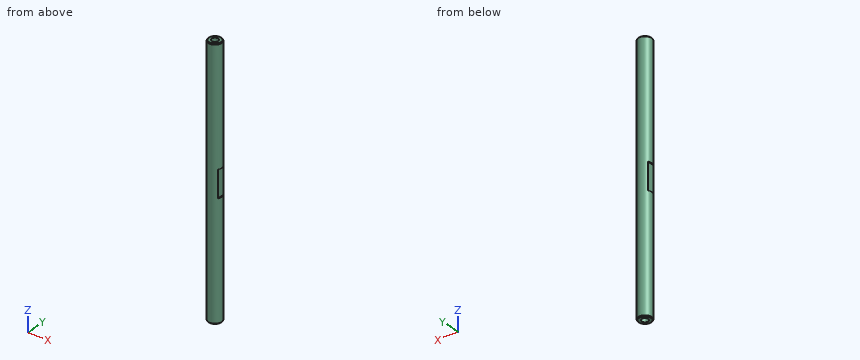
```python
from build123d import *

# Parameters (mm, degrees)
SKETCH_1_R             = 5
EXTRUDE_1_DEPTH        = 97
CUT_EXTRUDE_1_DEPTH    = 10
HOLE_WIZARD_M6_1_D     = 5
HOLE_WIZARD_M6_1_DEPTH = 15
HOLE_WIZARD_M6_1_TIP   = 1.502151548
HOLE_WIZARD_M6_2_D     = 5
HOLE_WIZARD_M6_2_DEPTH = 15
HOLE_WIZARD_M6_2_TIP   = 1.502151548
CHAMFER_1_SIZE         = 0.5


with BuildPart() as part:
    # 草图1 → 凸台-拉伸1 (new, symmetric)
    with BuildSketch(Plane.XY):
        with Locations(Location((0, 0, 0), (0, 0, 180))):
            Circle(SKETCH_1_R)
    extrude(amount=EXTRUDE_1_DEPTH, both=True)

    # 草图2 → 切除-拉伸1 (cut, symmetric)
    with BuildSketch(Plane.XY):
        with BuildLine():
            Line((-4.25, 2.633913438), (-4.25, -2.633913438))
            ThreePointArc((-4.25, -2.633913438), (-5, 0), (-4.25, 2.633913438))
        make_face()
        with BuildLine():
            Line((4.25, 2.633913438), (4.25, -2.633913438))
            ThreePointArc((4.25, -2.633913438), (5, 0), (4.25, 2.633913438))
        make_face()
    extrude(amount=CUT_EXTRUDE_1_DEPTH, both=True, mode=Mode.SUBTRACT)

    # M6 螺纹孔1
    with Locations(Plane.XY.offset(97)):
        with Locations((0, 0)):
            Hole(HOLE_WIZARD_M6_1_D / 2, depth=HOLE_WIZARD_M6_1_DEPTH)
            with Locations((0, 0, -(HOLE_WIZARD_M6_1_DEPTH + HOLE_WIZARD_M6_1_TIP / 2))):  # 118° drill point
                Cone(0, HOLE_WIZARD_M6_1_D / 2, HOLE_WIZARD_M6_1_TIP, mode=Mode.SUBTRACT)

    # M6 螺纹孔2
    with Locations(Plane(origin=(0, 0, -97), x_dir=(-1, 0, 0), z_dir=(0, 0, -1))):
        with Locations((0, 0)):
            Hole(HOLE_WIZARD_M6_2_D / 2, depth=HOLE_WIZARD_M6_2_DEPTH)
            with Locations((0, 0, -(HOLE_WIZARD_M6_2_DEPTH + HOLE_WIZARD_M6_2_TIP / 2))):  # 118° drill point
                Cone(0, HOLE_WIZARD_M6_2_D / 2, HOLE_WIZARD_M6_2_TIP, mode=Mode.SUBTRACT)

    # 倒角1
    chamfer_1_edges = [part.edges().sort_by_distance(p)[0] for p in [
        (5, 0, -97),
        (5, 0, 97),
    ]]
    chamfer(chamfer_1_edges, length=CHAMFER_1_SIZE)


solid = part.part
```
Here's how the part is built. I have some questions about the finished solid (model axes, mm). Give positions to 0.01 mm unless a question says otherwise; leave off trailing zeros. Order: outer loops, then holes, each group sorted by start corner. A loop starts at its lowest first (then second) coordinate and runs counter-clockwise, first axis right, second up. Notation, with made-up numbers: (-12.5, 13) -> (18.5, 13) arc R28 cw to (18.5, 41) -> close; hole circle Ø4 at (11.25, 14). An arc over 180 degrees is marked (long way). Use CSV: the item, a comma, the result in double quotes. Start each with the question number.
Item 1: I'm going to push flat-ended pins straight in: P1, Ø2.5, axis at y = -0.5, z = 2, coming from the +X side; P2, Ø0.6, axis at x = 5, y = -0.5, coming from the +Z side; P3, Ø2, axis at x = -2, z = 15.5, coming from the +Y side. Where does each tip first touch, or does it pass through?
Item 2: If I drill on probe 1 along Y at (x, z) = (0, 90.5); probe 2 along X at (y, z) = (4.25, -25.5), over which ranges is the centre line in solid material (lowest first)? Write a range as [from, to].
Item 3: Suppose I cut it at B-B (z = -68.5). List the corners of the cut face in (x, y) for me, and give its area (3 significant figures).
Item 4: Suppose I cut it at A-A (z = 4.5). List the corners of the cut face in (x, y) for me, and give its area (3 significant figures).
Answer block:
1,P1,"stops at x = 4.25"
1,P2,"stops at z = 96.78"
1,P3,"stops at y = 4.9"
2,probe 1,"y = [-5, -2.5], [2.5, 5]"
2,probe 2,"x = [-2.63, 2.63]"
3,outline,"circle Ø10 at (0, 0)"
3,area,"78.5 mm^2"
4,outline,"(-4.25, -2.63) arc R5 ccw to (4.25, -2.63) -> (4.25, 2.63) arc R5 ccw to (-4.25, 2.63) -> close"
4,area,"73.2 mm^2"
